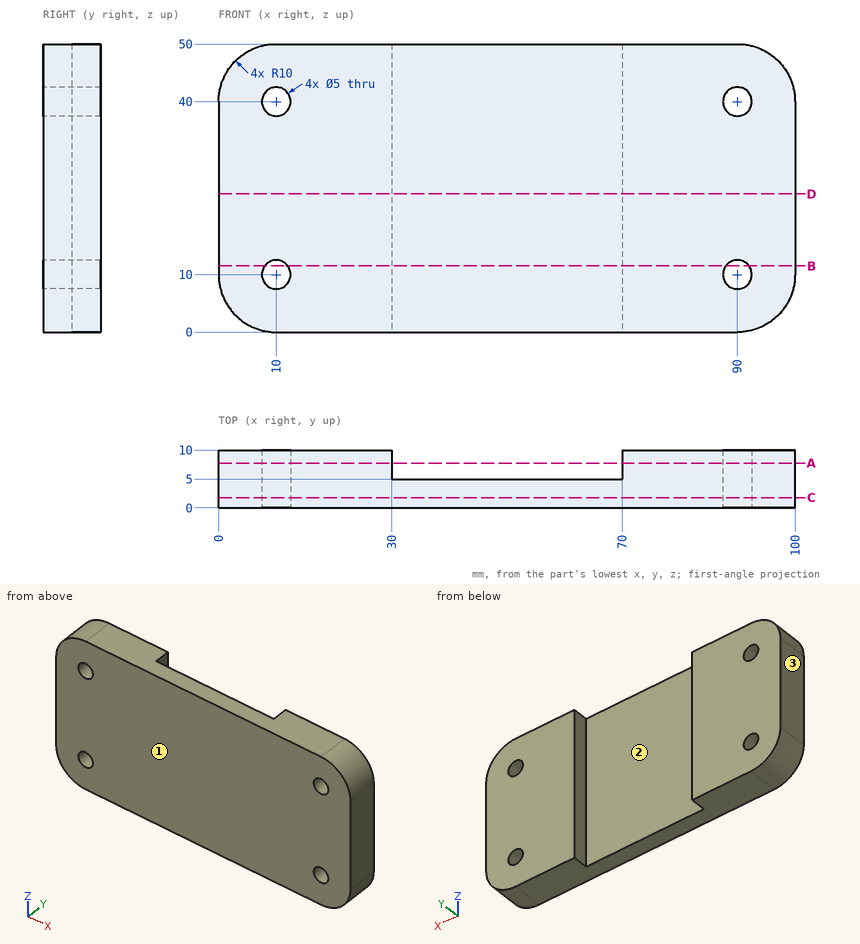
Here's the drawing with two shaded views (mm, measured from the low corner). I have some questions. Give positions to 0.01 mm unless a question says otherwise; leave off trailing zeros. Write each loop counter-clockwise with the first axis right and the second up, starting at its lowest first coordinate (ties: lowest second). Pieces come first, ordered by that corner, then holes. Notation, with made-up numbers: (-15.5, 78.25) -> (3.5, 78.25) arc R22 ccw to (3.5, 90.25) -> close; hole circle Ø5 at (-30, 69.5). An arc over 180 degrees is marked (long way). Use one line per item in the form item = value. Start each with the question number.
1. Imagine slicing it at D-D on z = 24. List the corners of the cut face in (x, y) for me, plus the area to 3 significant figures.
2. Thinking about a two-plate mould opening in X: for the marked faces 1, 2 and 3, which applies, +X half, -X half, draft (parallel to the pull), parting line (faces both ways), or undercut?
3. If I drill on L1, parallel to X at y = 6, z = 10; L2, parallel to X at y = 2.75, z = 10; L3, parallel to X at y = 6.75, z = 39, over which ranges is the centre line in solid material (lowest first)?
4. Imagine slicing it at B-B on z = 11.5. List the corners of the cut face in (x, y) for me, plus the area to 3 significant figures.
5. Will this pin go through, and if not, where does the flat tip stop? pin 1 Ø8 at (x, z) = (46, 32.5) entering from +Y.
6. Imagine slicing it at A-A on y = 7.75. List the corners of the cut face in (x, z) for me.
7. Imagine slicing it at C-C on y = 1.75. List the corners of the cut face in (x, z) for me, plus the area to 3 significant figures.
Entries:
q1.outline = (0, 0) -> (100, 0) -> (100, 10) -> (70, 10) -> (70, 5) -> (30, 5) -> (30, 10) -> (0, 10) -> close
q1.area = 800 mm²
q2.face_1 = draft
q2.face_2 = undercut
q2.face_3 = -X half
q3.L1 = 0 to 7.5, 12.5 to 30, 70 to 87.5, 92.5 to 100
q3.L2 = 0 to 7.5, 12.5 to 87.5, 92.5 to 100
q3.L3 = 0 to 7.71, 12.29 to 30, 70 to 87.71, 92.29 to 100
q4.outline = (0, 0) -> (8, 0) -> (8, 10) -> (0, 10) -> close; (12, 0) -> (88, 0) -> (88, 10) -> (70, 10) -> (70, 5) -> (30, 5) -> (30, 10) -> (12, 10) -> close; (92, 0) -> (100, 0) -> (100, 10) -> (92, 10) -> close
q4.area = 720 mm²
q5.pin_1 = 5
q6.outline = (0, 10) arc R10 ccw to (10, 0) -> (30, 0) -> (30, 50) -> (10, 50) arc R10 ccw to (0, 40) -> close; (70, 0) -> (90, 0) arc R10 ccw to (100, 10) -> (100, 40) arc R10 ccw to (90, 50) -> (70, 50) -> close; hole circle Ø5 at (10, 10); hole circle Ø5 at (10, 40); hole circle Ø5 at (90, 10); hole circle Ø5 at (90, 40)
q7.outline = (0, 10) arc R10 ccw to (10, 0) -> (90, 0) arc R10 ccw to (100, 10) -> (100, 40) arc R10 ccw to (90, 50) -> (10, 50) arc R10 ccw to (0, 40) -> close; hole circle Ø5 at (10, 10); hole circle Ø5 at (10, 40); hole circle Ø5 at (90, 10); hole circle Ø5 at (90, 40)
q7.area = 4,840 mm²
